```python
from build123d import *

# Parameters (mm, degrees)
BOSS_EXTRUDE1_DEPTH       = 8
M12_CLEARANCE_HOLE1_D     = 13.5
M12_CLEARANCE_HOLE1_DEPTH = 60
M12_CLEARANCE_HOLE1_TIP   = 4.055809178


with BuildPart() as part:
    # Sketch1 → Boss-Extrude1 (new body)
    with BuildSketch(Plane(origin=(0, 0, 0), x_dir=(1, 0, 0), z_dir=(0, 1, 0))):
        Polygon((0, 0), (100, 0), (100, 40), (40, 100), (0, 100), align=None)
    extrude(amount=BOSS_EXTRUDE1_DEPTH)

    # M12 Clearance Hole1
    with Locations(Plane(origin=(0, 8, 0), x_dir=(1, 0, 0), z_dir=(0, 1, 0))):
        with Locations((50, 50)):
            Hole(M12_CLEARANCE_HOLE1_D / 2, depth=M12_CLEARANCE_HOLE1_DEPTH)
            with Locations((0, 0, -(M12_CLEARANCE_HOLE1_DEPTH + M12_CLEARANCE_HOLE1_TIP / 2))):  # 118° drill point
                Cone(0, M12_CLEARANCE_HOLE1_D / 2, M12_CLEARANCE_HOLE1_TIP, mode=Mode.SUBTRACT)


solid = part.part
```
Source: CAD feature listing. Evaluate the final solid. Frame: model axes, mm. Give positions to 0.01 mm unless a question says otherwise; leave off trailing zeros. Loops run counter-clockwise (first coordinate to the right, second up) from the corner with the lowest first, then second, coordinate; pieces in that order, holes last. Notation, with made-up numbers: (-4, 73) -> (16, 73) arc R12 cw to (16, 78) -> close; hole circle Ø11 at (48.25, 13). An arc over 180 degrees is marked (long way). Use a Markdown table: item, result. Add a question column.
(1) Pull-direction query (X, two-part tool) for faces 1 (the face through (100, 4, -20)), 2 (the face through (20, 4, -100)), 3 (the face through (56.743, 3.944, -50.297)); classes: +X half, -X half, draft (parallel to the pull), parting line (faces both ways), or undercut.
(2) Section query A-A (x = 50). Output: boundary loops of the cut face in (y, z).
(3) Ray query, line 1 (Z direction, x = 50, y = 4.25); line 2 (X direction, y = 1.5, z = -50); line 3 (X direction, y = 4.75, z = -45). Return the intervals inside material, ascending.
(4) Section query B-B (z = -50). Output: boundary loops of the cut face in (x, y).
(5) Section query C-C (y = 4). Output: boundary loops of the cut face in (x, z).
(6) Section query D-D (z = -69.5). Output: boundary loops of the cut face in (x, y), then the cut area to 3 significant figures.
Checked values:
| question | item | result |
|---|---|---|
| 1 | face 1 | +X half |
| 1 | face 2 | draft |
| 1 | face 3 | undercut |
| 2 | outline | (0, -90) -> (8, -90) -> (8, -56.75) -> (0, -56.75) -> close; (0, -43.25) -> (8, -43.25) -> (8, 0) -> (0, 0) -> close |
| 3 | line 1 | -90 to -56.75, -43.25 to 0 |
| 3 | line 2 | 0 to 43.25, 56.75 to 90 |
| 3 | line 3 | 0 to 45.47, 54.53 to 95 |
| 4 | outline | (0, 0) -> (43.25, 0) -> (43.25, 8) -> (0, 8) -> close; (56.75, 0) -> (90, 0) -> (90, 8) -> (56.75, 8) -> close |
| 5 | outline | (0, -100) -> (40, -100) -> (100, -40) -> (100, 0) -> (0, 0) -> close; hole circle Ø13.5 at (50, -50) |
| 6 | outline | (0, 0) -> (70.5, 0) -> (70.5, 8) -> (0, 8) -> close |
| 6 | area | 564 mm^2 |
